Read the model definition and answer for the solid it produces. Units are mm, in the model's axes. Coordinates: 2 decimals unless noted, no trailing zeros. Write each loop counter-clockwise with the first axis right and the second up, starting at its lowest first coordinate (ties: lowest second). Pieces come first, ordered by that corner, then holes.
1) Find the intervals of material crossed by line 1 (X direction, y = 37, z = 321), in increasing order.
2) The part is cut by section A-A (y = 17.5). Determine the outline of the cut face in (x, z), then the cut area to 3 significant figures.
3) The part is cut by section C-C (z = 226). Determine the outline of the cut face in (x, y), then the cut area to 3 significant figures.
from build123d import *

# Parameters (mm, degrees)
SKETCH_1_W          = 50
SKETCH_1_H          = 50
SKETCH_1_W_2        = 44
SKETCH_1_H_2        = 44
EXTRUDE_1_DEPTH     = 600
SKETCH_2_W          = 50
SKETCH_2_H          = 50
SKETCH_2_W_2        = 44
SKETCH_2_H_2        = 44
CUT_EXTRUDE_1_DEPTH = 25


with BuildPart() as part:
    # 草图1 → 凸台-拉伸1 (new body)
    with BuildSketch(Plane.XY):
        with Locations((25, 25)):
            Rectangle(SKETCH_1_W, SKETCH_1_H)
        with Locations((25, 25)):
            Rectangle(SKETCH_1_W_2, SKETCH_1_H_2, mode=Mode.SUBTRACT)
    extrude(amount=EXTRUDE_1_DEPTH)

    # 草图2 → 切除-拉伸1 (cut)
    with BuildSketch(Plane.XY.offset(600)):
        with Locations((25, 25)):
            Rectangle(SKETCH_2_W, SKETCH_2_H)
        with Locations((25, 25)):
            Rectangle(SKETCH_2_W_2, SKETCH_2_H_2, mode=Mode.SUBTRACT)
    extrude(amount=-CUT_EXTRUDE_1_DEPTH, mode=Mode.SUBTRACT)


solid = part.part
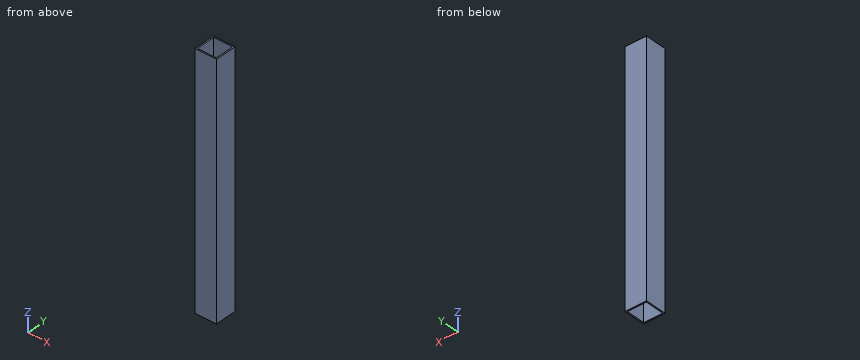
Reported:
1. line 1: x = 0 to 3, 47 to 50
2. outline: (0, 0) - (3, 0) - (3, 575) - (0, 575) - close; (47, 0) - (50, 0) - (50, 575) - (47, 575) - close
2. area: 3,450 mm2
3. outline: (0, 0) - (50, 0) - (50, 50) - (0, 50) - close; hole (3, 3) - (47, 3) - (47, 47) - (3, 47) - close
3. area: 564 mm2
